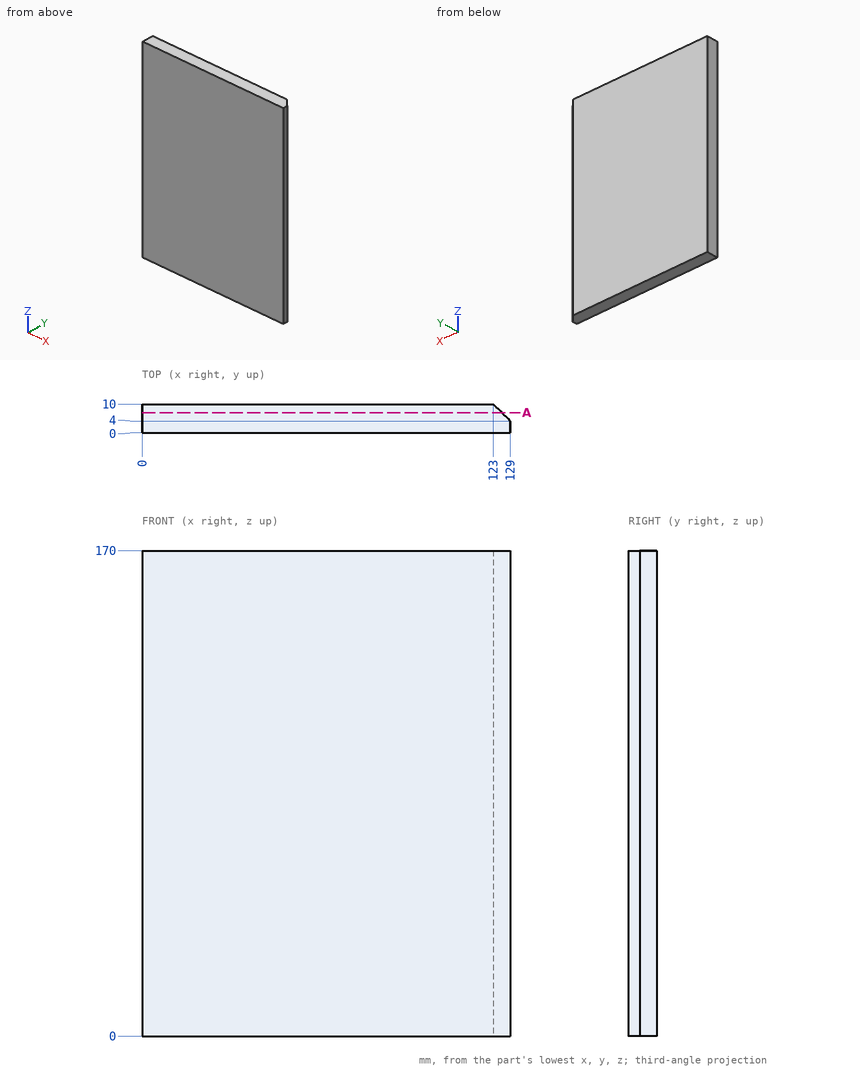
Geometry check sheet. Reference: drawing and pictorial views, mm from the part's lowest x, y, z. Give positions to 0.01 mm unless a question says otherwise; leave off trailing zeros. Order: outer loops, then holes, each group sorted by start corner. A loop starts at its lowest first (then second) coordinate and runs counter-clockwise, first axis right, second up. Notation, with made-up numbers: M 48,-13.75 L 86,-13.75 A17 cw 86,13.25 Z; hole C 73,52.25 d3. An arc over 180 degrees is marked long. Answer in a Markdown table with one row per item. Add a question column.
Item 1: Gauge pin test, flat ends, axial feed: pin 1 (12 mm diameter, centred on x = 89, z = 84.5, fed in from -Y); pin 2 (2 mm diameter, centred on y = 8, z = 20, fed in from +X). Record the tip position at first contact, or that the pin passes through.
Item 2: Section check A-A, the plane y = 7. Enter the section's corners in (x, z).
Item 3: Scan lines: probe 1 along X at (y, z) = (9, 59.5); probe 2 along X at (y, z) = (7.75, 139). Record each from-to range of solid material in increasing order. Write a range as from..to.
Filled sheet:
| question | item | result |
|---|---|---|
| 1 | pin 1 | stops at y = 0 |
| 1 | pin 2 | stops at x = 126 |
| 2 | outline | M 0,0 L 126,0 L 126,170 L 0,170 Z |
| 3 | probe 1 | x = 0..124 |
| 3 | probe 2 | x = 0..125.25 |
